from build123d import *

# Parameters (mm, degrees)
SKETCH1_W           = 100
SKETCH1_H           = 90
SKETCH1_R           = 24
BOSS_EXTRUDE1_DEPTH = 65


with BuildPart() as part:
    # Sketch1 → Boss-Extrude1 (new body)
    with BuildSketch(Plane.XY):
        with Locations((50, 45)):
            Rectangle(SKETCH1_W, SKETCH1_H)
        with Locations((50, 45)):
            Circle(SKETCH1_R, mode=Mode.SUBTRACT)
    extrude(amount=BOSS_EXTRUDE1_DEPTH)


solid = part.part
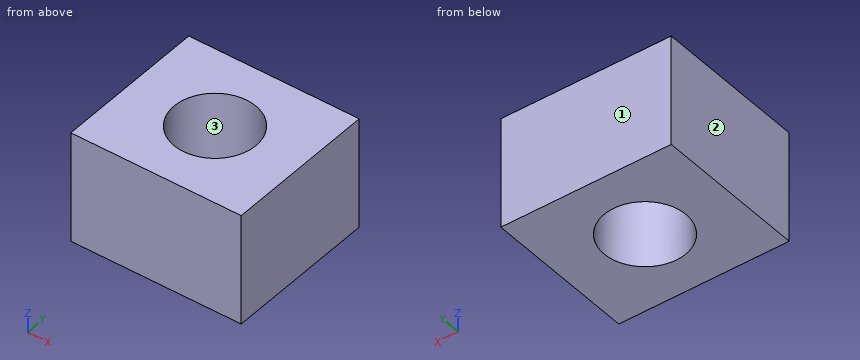
Geometry: final body of the model. Coordinates: model frame, mm. Face numbers are marked on the shaded views. Coordinates: 2 decimals unless noted, no trailing zeros. Order: outer loops, then holes, each group sorted by start corner. A loop starts at its lowest first (then second) coordinate and runs counter-clockwise, first axis right, second up. Notation, with made-up numbers: M -7.75,13.5 L 18.25,13.5 A20 cw 18.25,52.5 Z; hole C 22,43.5 d7. An arc over 180 degrees is marked long. One line per question, with ' | ' between items. Start each with the question number.
Item 1: Ray query, probe 1 along Y at (x, z) = (50, 25.5); probe 2 along Y at (x, z) = (39.5, 38); probe 3 along X at (y, z) = (44.5, 21.5). Return the intervals inside material, ascending. Write a range as [from, to].
Item 2: Cut plane C-C, the plane y = 45. Return the cut outline in (x, z).
Item 3: Cut plane A-A, the plane x = 50. Return the cut outline in (y, z).
Item 4: Cut plane B-B, the plane z = 52. Return the cut outline in (x, y).
Item 5: Draft query along Y for the marked faces 1, 2 and 3. Return one class per face: released by +Y, released by -Y, zero draft, split by the parting line, or undercut.
A:
1) probe 1: y = [0, 21], [69, 90] | probe 2: y = [0, 23.42], [66.58, 90] | probe 3: x = [0, 26.01], [73.99, 100]
2) outline: M 0,0 L 26,0 L 26,65 L 0,65 Z; M 74,0 L 100,0 L 100,65 L 74,65 Z
3) outline: M 0,0 L 21,0 L 21,65 L 0,65 Z; M 69,0 L 90,0 L 90,65 L 69,65 Z
4) outline: M 0,0 L 100,0 L 100,90 L 0,90 Z; hole C 50,45 d48
5) face 1: released by +Y | face 2: zero draft | face 3: undercut
